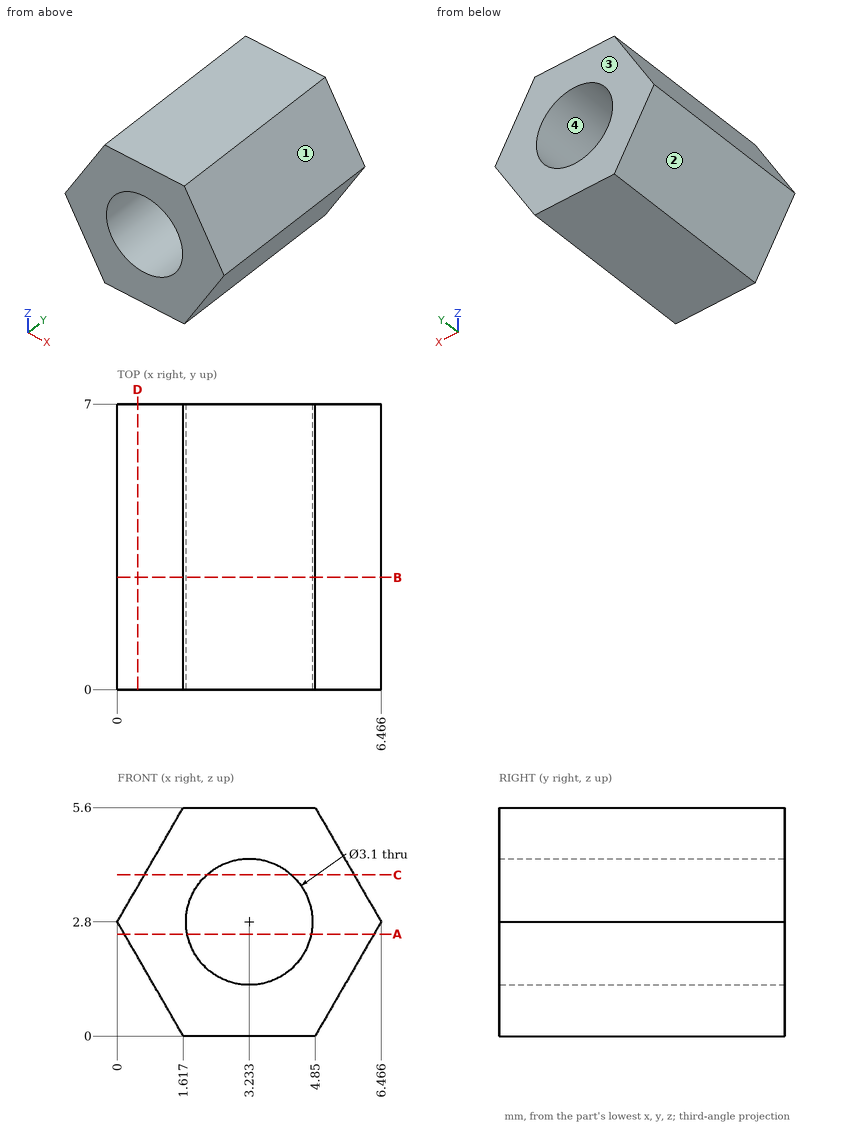
For this review, use the dimensioned drawing (mm, ordinates from the lowest corner) and the shaded views. Coordinates: 2 decimals unless noted, no trailing zeros. Loops run counter-clockwise (first coordinate to the right, second up) from the corner with the lowest first, then second, coordinate; pieces in that order, holes last. Notation, with made-up numbers: (62.5, -35) - (104.5, -35) arc R16 cw to (104.5, -10) - close; hole circle Ø1 at (70.25, 60). An arc over 180 degrees is marked (long way). Use CSV: the item, a comma, the result in double quotes. Start each with the question number.
1) Wall thickness on L1, parallel to Z at x = 3.75, y = 4; L2, parallel to X at y = 6.5, z = 2.65 (1 decimal); L3, parallel to Z at x = 2, y = 5: over which ranges is each line inside the solid? List them lowest first. Write a range as from..to.
2) Consider section A-A on z = 2.5. Write out the cut boundary in (x, y).
3) Consider section C-C on z = 3.95. Write out the cut boundary in (x, y), then the cut area to 3 significant figures.
4) Consider section B-B on y = 2.75. Write out the cut boundary in (x, z).
5) Consider section D-D on x = 0.5. Write out the cut boundary in (y, z), then the cut area to 3 significant figures.
6) The part is to be moulded in two halves that separate along X. For the marked faces 1, 2, 3 and 4, say which applies: +X half, -X half, draft (parallel to the pull), parting line (faces both ways), or undercut.
Geometry says:
1,L1,"0..1.34, 4.26..5.6"
1,L2,"0.1..1.7, 4.8..6.4"
1,L3,"0..1.86, 3.74..5.6"
2,outline,"(0.17, 0) - (1.71, 0) - (1.71, 7) - (0.17, 7) - close; (4.75, 0) - (6.29, 0) - (6.29, 7) - (4.75, 7) - close"
3,outline,"(0.66, 0) - (2.19, 0) - (2.19, 7) - (0.66, 7) - close; (4.27, 0) - (5.8, 0) - (5.8, 7) - (4.27, 7) - close"
3,area,"21.4 mm^2"
4,outline,"(0, 2.8) - (1.62, 0) - (4.85, 0) - (6.47, 2.8) - (4.85, 5.6) - (1.62, 5.6) - close; hole circle Ø3.1 at (3.23, 2.8)"
5,outline,"(0, 1.93) - (7, 1.93) - (7, 3.67) - (0, 3.67) - close"
5,area,"12.1 mm^2"
6,face 1,"+X half"
6,face 2,"-X half"
6,face 3,"draft"
6,face 4,"undercut"
